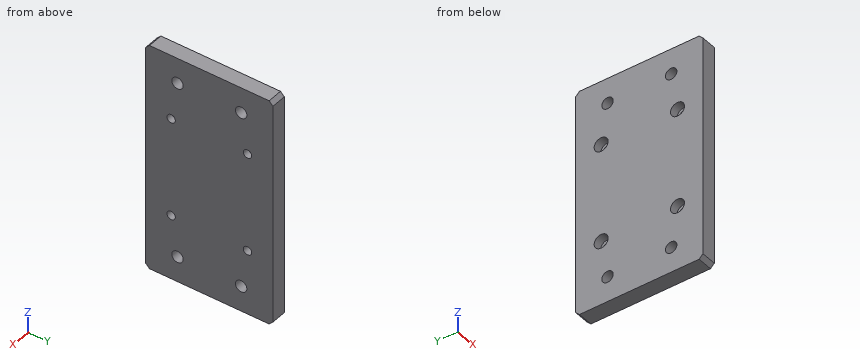
```python
from build123d import *

# Parameters (mm, degrees)
SKETCH_1_W                = 180
SKETCH_1_H                = 100
EXTRUDE_1_DEPTH           = 12
HOLE_WIZARD_1_D           = 6.6
HOLE_WIZARD_1_CBORE_D     = 11
HOLE_WIZARD_1_CBORE_DEPTH = 6.8
HOLE_WIZARD_9_0_9_1_D     = 9
CHAMFER_1_SIZE            = 3


with BuildPart() as part:
    # 草图1 → 凸台-拉伸1 (new body)
    with BuildSketch(Plane(origin=(0, 0, 0), x_dir=(0, 0, -1), z_dir=(1, 0, 0))):
        Rectangle(SKETCH_1_W, SKETCH_1_H)
    extrude(amount=EXTRUDE_1_DEPTH)

    # 打孔尺寸(%根据)内六角圆柱头螺钉的类型1 (through all)
    with Locations(Plane.ZY):
        with Locations((-39, 30), (-39, -30), (39, 30), (39, -30)):
            CounterBoreHole(HOLE_WIZARD_1_D / 2, HOLE_WIZARD_1_CBORE_D / 2, HOLE_WIZARD_1_CBORE_DEPTH)

    # Ø9.0 (9) 直径孔1 (through all)
    with Locations(Plane.ZY):
        with Locations((-70, 25), (-70, -25), (70, 25), (70, -25)):
            Hole(HOLE_WIZARD_9_0_9_1_D / 2)

    # 倒角1
    chamfer_1_edges = [part.edges().sort_by_distance(p)[0] for p in [
        (6, -50, -90),
        (6, -50, 90),
        (6, 50, 90),
        (6, 50, -90),
    ]]
    chamfer(chamfer_1_edges, length=CHAMFER_1_SIZE)


solid = part.part
```
Can you work these out from the model? Positions are in its coordinate system, mm. Coordinates: 2 decimals unless noted, no trailing zeros. Loops run counter-clockwise (first coordinate to the right, second up) from the corner with the lowest first, then second, coordinate; pieces in that order, holes last. Notation, with made-up numbers: (53.25, 78) - (64.25, 78) arc R21 ccw to (64.25, 112) - close; hole circle Ø7 at (11.25, 28). An arc over 180 degrees is marked (long way). Answer as CSV lines item,"result". Start each with the question number.
1) Suppose I cut it at C-C (z = 39). Please give me the cut outline in (x, y).
2) Suppose I cut it at A-A (x = 3.75). Count the separate pieces of the cut face and the enclosed holes in it, plus the area to 3 significant figures.
3) Suppose I cut it at B-B (z = -70). Please give me the cut outline in (x, y), plus the area to 3 significant figures.
4) I need wall thicknesses on line 1 (Y direction, x = 3.75, z = 39); line 2 (Y direction, x = 5, z = 70); line 3 (Z direction, x = 11, y = -23.5). Which ranges of each line are inside material? Lowest first, please. Write a range as from..to.
5) For pin 1 (17.5 mm diameter, centred on y = -30, z = 39, fed in from +X); pin 2 (6 mm diameter, centred on y = 25, z = -71, fed in from -X); pin 3 (8.5 mm diameter, centred on y = 30, z = 39, fed in from -X), each with a flat end and sliding along its axis, tell me the tip position at first contact or that it passes through.
Check result:
1,outline,"(0, -50) - (12, -50) - (12, -33.3) - (6.8, -33.3) - (6.8, -35.5) - (0, -35.5) - close; (0, -24.5) - (6.8, -24.5) - (6.8, -26.7) - (12, -26.7) - (12, 26.7) - (6.8, 26.7) - (6.8, 24.5) - (0, 24.5) - close; (0, 35.5) - (6.8, 35.5) - (6.8, 33.3) - (12, 33.3) - (12, 50) - (0, 50) - close"
2,separate pieces,"1"
2,enclosed holes,"8"
2,area,"17,300 mm²"
3,outline,"(0, -50) - (12, -50) - (12, -29.5) - (0, -29.5) - close; (0, -20.5) - (12, -20.5) - (12, 20.5) - (0, 20.5) - close; (0, 29.5) - (12, 29.5) - (12, 50) - (0, 50) - close"
3,area,"984 mm²"
4,line 1,"y = -50..-35.5, -24.5..24.5, 35.5..50"
4,line 2,"y = -50..-29.5, -20.5..20.5, 29.5..50"
4,line 3,"z = -90..-74.24, -65.76..65.76, 74.24..90"
5,pin 1,"stops at x = 12"
5,pin 2,"passes through"
5,pin 3,"stops at x = 6.8"
